```python
from build123d import *

# Parameters (mm, degrees)
SKETCH1_R           = 29
BOSS_EXTRUDE1_DEPTH = 25
SKETCH2_R           = 27
BOSS_EXTRUDE2_DEPTH = 100
SKETCH7_R           = 24
CUT_EXTRUDE4_DEPTH  = 22
SKETCH8_R           = 24.1
CUT_EXTRUDE5_DEPTH  = 3
CHAMFER1_SIZE       = 1
SKETCH9_R           = 18
CUT_EXTRUDE6_DEPTH  = 18
SKETCH10_R          = 18.25
CUT_EXTRUDE7_DEPTH  = 2
CHAMFER2_SIZE       = 1


with BuildPart() as part:
    # Sketch1 → Boss-Extrude1 (new body)
    with BuildSketch(Plane.XY):
        Circle(SKETCH1_R)
    extrude(amount=BOSS_EXTRUDE1_DEPTH)

    # Sketch2 → Boss-Extrude2 (add)
    with BuildSketch(Plane.XY.offset(25)):
        Circle(SKETCH2_R)
    extrude(amount=BOSS_EXTRUDE2_DEPTH)

    # Sketch7 → Cut-Extrude4 (cut)
    with BuildSketch(Plane(origin=(0, 0, 0), x_dir=(-1, 0, 0), z_dir=(0, 0, -1))):
        Circle(SKETCH7_R)
    extrude(amount=-CUT_EXTRUDE4_DEPTH, mode=Mode.SUBTRACT)

    # Sketch8 → Cut-Extrude5 (cut)
    with BuildSketch(Plane(origin=(0, 0, 22), x_dir=(-1, 0, 0), z_dir=(0, 0, -1))):
        Circle(SKETCH8_R)
    extrude(amount=-CUT_EXTRUDE5_DEPTH, mode=Mode.SUBTRACT)

    # Chamfer1
    chamfer1_edges = [part.edges().sort_by_distance(p)[0] for p in [
        (24, 0, 0),
    ]]
    chamfer(chamfer1_edges, length=CHAMFER1_SIZE)

    # Sketch9 → Cut-Extrude6 (cut)
    with BuildSketch(Plane.XY.offset(125)):
        Circle(SKETCH9_R)
    extrude(amount=-CUT_EXTRUDE6_DEPTH, mode=Mode.SUBTRACT)

    # Sketch10 → Cut-Extrude7 (cut)
    with BuildSketch(Plane.XY.offset(107)):
        Circle(SKETCH10_R)
    extrude(amount=-CUT_EXTRUDE7_DEPTH, mode=Mode.SUBTRACT)

    # Chamfer2
    chamfer2_edges = [part.edges().sort_by_distance(p)[0] for p in [
        (-18, 0, 125),
    ]]
    chamfer(chamfer2_edges, length=CHAMFER2_SIZE)


solid = part.part
```
CAD build for the part. Positions are in the model's coordinates, mm. A direction names the side the tool comes from. Round coordinates to 2 decimals unless told otherwise and drop trailing zeros. Order: outer loops, then holes, each group sorted by start corner. A loop starts at its lowest first (then second) coordinate and runs counter-clockwise, first axis right, second up. Notation, with made-up numbers: (-34, 2) - (2, 2) arc R24 cw to (2, 34) - close; hole circle Ø11 at (-6.5, -9). An arc over 180 degrees is marked (long way). Use CSV: the item, a comma, the result in double quotes. Start each with the question number.
1) Tool access for faces 4 (the flat face through (13, 22, 0)), 5 (the cylindrical face through (13.38, -25.73, 12.32)), 6 (the cylindrical face through (17.76, 16.29, 23.48)), 7 (the cylindrical face through (-2.343, 17.847, 115.619)), 8 (the cylindrical face through (23.977, 1.055, 11.353)): list every direction of +Z, -Z, +X, -X, +Y, -Y with a clear straight run to the whole face (end or side of a thin tool).
2) Pin check, flat tips, straight feed: pin 1 Ø2 at (x, z) = (-9, 58.5) entering from +Y; pin 2 Ø10 at (y, z) = (-18, 112) entering from -X; pin 3 Ø8 at (y, z) = (-16, 55.5) entering from -X. Stop position of each tip, or through.
3) Saw through at A-A (x = 0). List the corners of the cut face in (y, z), and give its area (3 significant figures).
4) Saw through at C-C (z = 100). List the corners of the cut face in (x, y), and give its area (3 significant figures).
5) Two-plate mould, pull along X, no slides. Class faces 1 (the cylindrical face through (-5.85, -26.36, 74.3)), 2 (the flat face through (5.6, 18.4, 125)), 3 (the flat face through (0, 0, 105)): pulls with the +X half, pulls with the -X half, needs draft (parallel to the pull), parting line crosses it, or undercut.
6) Wall check: L1, parallel to Y at x = 0, z = 22.95; L2, parallel to Z at x = -26.5, y = -8; L3, parallel to Z at x = -16, y = -14. Give the ranges that are in metal, low to high. Write a range as [from, to].
Values follow:
1,face 4,"-Z, +X, -X, +Y, -Y"
1,face 5,"+Z, -Z"
1,face 6,"none"
1,face 7,"+Z"
1,face 8,"-Z"
2,pin 1,"stops at y = 25.79"
2,pin 2,"stops at x = -23.66"
2,pin 3,"stops at x = -24.19"
3,outline,"(-29, 0) - (-25, 0) - (-24, 1) - (-24, 22) - (-24.1, 22) - (-24.1, 25) - (24.1, 25) - (24.1, 22) - (24, 22) - (24, 1) - (25, 0) - (29, 0) - (29, 25) - (27, 25) - (27, 125) - (19, 125) - (18, 124) - (18, 107) - (18.25, 107) - (18.25, 105) - (-18.25, 105) - (-18.25, 107) - (-18, 107) - (-18, 124) - (-19, 125) - (-27, 125) - (-27, 25) - (-29, 25) - close"
3,area,"4,930 mm2"
4,outline,"circle Ø54 at (0, 0)"
4,area,"2,290 mm2"
5,face 1,"parting line crosses it"
5,face 2,"needs draft"
5,face 3,"undercut"
6,L1,"y = [-29, -24.1], [24.1, 29]"
6,L2,"z = [0, 25]"
6,L3,"z = [25, 125]"
